from build123d import *

# Parameters (mm, degrees)
SKETCH_1_R      = 3.54
SKETCH_1_R_2    = 1.176
EXTRUDE_1_DEPTH = 4.5


with BuildPart() as part:
    # 草图1 → 凸台-拉伸1 (new body)
    with BuildSketch(Plane.XY):
        with BuildLine():
            Line((22, 3), (5.232070686, 3))
            ThreePointArc((5.232070686, 3), (-6.022909015, 0.314850207), (4.890755195, -3.529175156))
            ThreePointArc((4.890755195, -3.529175156), (10.083161164, 0.184396071), (16.464202545, 0))
            Line((16.464202545, 0), (19, 0))
            ThreePointArc((19, 0), (24.121320344, -2.121320344), (22, 3))
        make_face()
        Circle(SKETCH_1_R, mode=Mode.SUBTRACT)
        with Locations((22, 0)):
            Circle(SKETCH_1_R_2, mode=Mode.SUBTRACT)
    extrude(amount=EXTRUDE_1_DEPTH)


solid = part.part
Build history of the part. All positions in model axes, mm. A direction names the side the tool comes from. Give positions to 0.01 mm unless a question says otherwise; leave off trailing zeros. Order: outer loops, then holes, each group sorted by start corner. A loop starts at its lowest first (then second) coordinate and runs counter-clockwise, first axis right, second up. Notation, with made-up numbers: M 11.25,-28 L 50.25,-28 A10 cw 50.25,-9 Z; hole C 77.5,85.5 d5. An arc over 180 degrees is marked long. Use one line per item in the form item = value.
Q1. Which spindle directions (+Z, -Z, +X, -X, +Y, -Y) get a long thin tool onto all of the face, cutting with end or side? Do faces 1 (the flat face through (9, 0, 4.5)), 2 (the flat face through (18, 0, 2)). Say none if no direction does.
Conclusion:
face_1 = +Z, +X, -X, +Y, -Y
face_2 = +Z, -Z, -Y
Q2. Pin check, flat tips, straight feed: P1, Ø2, axis at x = 2, z = 0.5, coming from the -Y side; P2, Ø1.5, axis at x = 13.5, y = -0.5, coming from the +Z side; P3, Ø1.3, axis at x = 15.5, z = 3, coming from the +Y side; P4, Ø2, axis at x = -1.5, z = 1.5, coming from the -Y side. Stop position of each tip, or through.
Conclusion:
P1 = -5.95
P2 = through
P3 = 3
P4 = -6.01
Q3. Wall check: probe 1 along X at (y, z) = (-2.5, 3.35); probe 2 along X at (y, z) = (-2, 1.55); probe 3 along Y at (x, z) = (0, 3.65). Give the ranges that are in metal, low to high.
Conclusion:
probe_1 = -5.49 to -2.51, 2.51 to 5.74, 20.34 to 23.66
probe_2 = -5.69 to -2.92, 2.92 to 6.25, 19.76 to 24.24
probe_3 = -6.03 to -3.54, 3.54 to 6.03
Q4. Slice it at C-C, the plane y = -2. Write the cut outline in (x, z), and give its area (3 significant figures).
Conclusion:
outline = M -5.69,0 L -2.92,0 L -2.92,4.5 L -5.69,4.5 Z; M 2.92,0 L 6.25,0 L 6.25,4.5 L 2.92,4.5 Z; M 19.76,0 L 24.24,0 L 24.24,4.5 L 19.76,4.5 Z
area = 47.6 mm2
Q5. Slice it at A-A, the plane x = 0. Write the cut outline in (y, z).
Conclusion:
outline = M -6.03,0 L -3.54,0 L -3.54,4.5 L -6.03,4.5 Z; M 3.54,0 L 6.03,0 L 6.03,4.5 L 3.54,4.5 Z
Q6. Pull direction Y, two halves, no side cores. Call faces 3 (the flat face through (14, 3, 2)), 4 (the cylindrical face through (3.377, 1.063, 2.218)), 5 (the cylindrical face through (24.05, -2.19, 2.22)), 6 (the cylindrical face through (20.825, 0.052, 2.218)): released by +Y, released by -Y, zero draft, split by the parting line, or undercut.
Conclusion:
face_3 = released by +Y
face_4 = undercut
face_5 = split by the parting line
face_6 = undercut
Q7. Slice it at B-B, the plane z = 1.95. Write the cut outline in (x, y), and give its area (3 significant figures).
Conclusion:
outline = M 4.89,-3.53 A10 cw 16.46,0 L 19,0 A3 ccw long 22,3 L 5.23,3 A6.03 ccw long Z; hole C 0,0 d7.08; hole C 22,0 d2.35
area = 141 mm2
Q8. Slice it at D-D, the plane x = -4. Write the cut outline in (y, z).
Conclusion:
outline = M -4.51,0 L 4.51,0 L 4.51,4.5 L -4.51,4.5 Z
